from build123d import *

# Parameters (mm, degrees)
EXTRUDE_THIN3_DEPTH = 14
CUT_EXTRUDE2_REACH  = 36.455
SKETCH3_R           = 2.25


with BuildPart() as part:
    # Sketch1 → Extrude-Thin3 (new body)
    with BuildSketch(Plane(origin=(0, 0, 0), x_dir=(1, 0, 0), z_dir=(0, 1, 0))):
        with BuildLine():
            Line((0, -30), (0, -18.940696925))
            ThreePointArc((0, -18.940696925), (-0.398266916, -17.922765586), (-1.381578947, -17.445378747))
            ThreePointArc((-1.381578947, -17.445378747), (-4.334524238, -16.954701402), (-7.160644531, -15.967941943))
            ThreePointArc((-7.160644531, -15.967941943), (-7.945976251, -15.140108401), (-7.921660959, -13.999291567))
            ThreePointArc((-7.921660959, -13.999291567), (-5, 0), (-7.921660959, 13.999291567))
            ThreePointArc((-7.921660959, 13.999291567), (-7.945976251, 15.140108401), (-7.160644531, 15.967941943))
            ThreePointArc((-7.160644531, 15.967941943), (-4.334524238, 16.954701402), (-1.381578947, 17.445378747))
            ThreePointArc((-1.381578947, 17.445378747), (-0.398266916, 17.922765586), (0, 18.940696925))
            Line((0, 18.940696925), (0, 30))
            Line((0, 30), (-1.5, 30))
            Line((-1.5, 30), (-1.5, 18.940696925))
            ThreePointArc((-1.5, 18.940696925), (-4.706054887, 18.407961522), (-7.774414062, 17.336622681))
            ThreePointArc((-7.774414063, 17.336622681), (-9.345077502, 15.680955597), (-9.296446918, 13.399321928))
            ThreePointArc((-9.296446918, 13.399321928), (-6.5, 0), (-9.296446918, -13.399321928))
            ThreePointArc((-9.296446918, -13.399321928), (-9.345077502, -15.680955597), (-7.774414062, -17.336622681))
            ThreePointArc((-7.774414063, -17.336622681), (-4.706054887, -18.407961522), (-1.5, -18.940696925))
            Line((-1.5, -18.940696925), (-1.5, -30))
            Line((-1.5, -30), (0, -30))
        make_face()
    extrude(amount=EXTRUDE_THIN3_DEPTH)

    # Sketch3 → Cut-Extrude2 (cut, up to next)
    with BuildSketch(Plane(origin=(0, 0, 0), x_dir=(0, 0, -1), z_dir=(1, 0, 0)), mode=Mode.PRIVATE) as cut_extrude2_sk1:
        with Locations((-24, 7)):
            Circle(SKETCH3_R)
    cut_extrude2_tool1 = extrude(cut_extrude2_sk1.sketch, amount=-CUT_EXTRUDE2_REACH, mode=Mode.PRIVATE) & part.part
    # Sketch3 → Cut-Extrude2 (cut, up to next)
    with BuildSketch(Plane(origin=(0, 0, 0), x_dir=(0, 0, -1), z_dir=(1, 0, 0)), mode=Mode.PRIVATE) as cut_extrude2_sk2:
        with Locations((24, 7)):
            Circle(SKETCH3_R)
    cut_extrude2_tool2 = extrude(cut_extrude2_sk2.sketch, amount=-CUT_EXTRUDE2_REACH, mode=Mode.PRIVATE) & part.part
    add(cut_extrude2_tool1.solids().sort_by_distance((0, 7, 24))[0], mode=Mode.SUBTRACT)
    add(cut_extrude2_tool2.solids().sort_by_distance((0, 7, -24))[0], mode=Mode.SUBTRACT)


solid = part.part
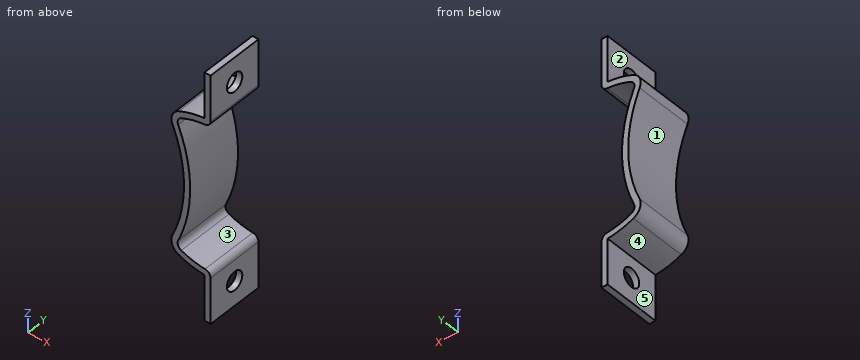
The listing builds one solid part. Answer for the finished solid, in the listing's coordinates (mm). Face numbers are marked on the shaded views. A direction names the side the tool comes from. Coordinates: 2 decimals unless noted, no trailing zeros. Write each loop counter-clockwise with the first axis right and the second up, starting at its lowest first coordinate (ties: lowest second). Pieces come first, ordered by that corner, then holes. Notation, with made-up numbers: M 21,-29.5 L 35,-29.5 A18 ccw 35,-0.5 Z; hole C 30,-39.75 d5. An arc over 180 degrees is marked long. Put each result on its own line as item: value. Start each with the question number.
1. Consider line 1 (Y direction, x = -0.5, z = 24); line 2 (X direction, y = 1.25, z = 22.5); line 3 (Z direction, x = -1.25, y = 2.5). Determine where each line is inside the solid, lowest interval first. Write a range as from..to.
2. Which of the six approach directions +Z, -Z, +X, -X, +Y, -Y give full straight-line access (tool end or side, diameter ignored) to the marked faces 1 and 2?
3. For a pull along Z with two mould halves and no side action, classify the marked faces 3, 4 and 5 as pulls with the +Z half, pulls with the -Z half, needs draft (parallel to the pull), parting line crosses it, or undercut.
4. A cutting plane is placed at D-D on y = 12.75. Write down the section's boundary in (x, z), then the cut area to 3 significant figures.
5. A cutting plane is placed at C-C on x = -3. Write down the section's boundary in (y, z), then the cut area to 3 significant figures.
6. A cutting plane is placed at A-A on z = -24. Write down the section's boundary in (x, y), then the cut area to 4 significant figures.
7. Flat-ended cylindrical pins translate along their axes: P1, Ø7, axis at y = 7, z = 24, coming from the -X side; P2, Ø1.5, axis at x = -4.5, z = 16, coming from the +Y side; P3, Ø2, axis at x = -7.5, y = 12, coming from the +Z side. Find the tip coordinate at first contact, or state that the pin passes through.
8. A cutting plane is placed at B-B on y = 7. Write down the section's boundary in (x, z), then the cut area to 3 significant figures.
Resolved:
1. line 1: y = 0..4.75, 9.25..14
1. line 2: x = -1.5..0
1. line 3: z = -30..-17.46, 17.46..30
2. face 1: -X, +Y, -Y
2. face 2: +Z, -X, +Y, -Y
3. face 3: undercut
3. face 4: pulls with the -Z half
3. face 5: needs draft
4. outline: M -9.3,-13.4 A3 ccw -7.77,-17.34 A19 ccw -1.5,-18.94 L -1.5,-30 L 0,-30 L 0,-18.94 A1.5 ccw -1.38,-17.45 A17.5 cw -7.16,-15.97 A1.5 cw -7.92,-14 A35 ccw -7.92,14 A1.5 cw -7.16,15.97 A17.5 cw -1.38,17.45 A1.5 ccw 0,18.94 L 0,30 L -1.5,30 L -1.5,18.94 A19 ccw -7.77,17.34 A3 ccw -9.3,13.4 A33.5 cw Z
4. area: 108 mm2
5. outline: M 0,-18.76 L 14,-18.76 L 14,-17.24 L 0,-17.24 Z; M 0,17.24 L 14,17.24 L 14,18.76 L 0,18.76 Z
5. area: 42.6 mm2
6. outline: M -1.5,0 L 0,0 L 0,4.75 L -1.5,4.75 Z; M -1.5,9.25 L 0,9.25 L 0,14 L -1.5,14 Z
6. area: 14.25 mm2
7. P1: stops at x = -1.5
7. P2: passes through
7. P3: stops at z = 17.85
8. outline: M -9.3,-13.4 A3 ccw -7.77,-17.34 A19 ccw -1.5,-18.94 L -1.5,-21.75 L 0,-21.75 L 0,-18.94 A1.5 ccw -1.38,-17.45 A17.5 cw -7.16,-15.97 A1.5 cw -7.92,-14 A35 ccw -7.92,14 A1.5 cw -7.16,15.97 A17.5 cw -1.38,17.45 A1.5 ccw 0,18.94 L 0,21.75 L -1.5,21.75 L -1.5,18.94 A19 ccw -7.77,17.34 A3 ccw -9.3,13.4 A33.5 cw Z; M -1.5,-30 L 0,-30 L 0,-26.25 L -1.5,-26.25 Z; M -1.5,26.25 L 0,26.25 L 0,30 L -1.5,30 Z
8. area: 94.6 mm2
